from build123d import *

# Parameters (mm, degrees)
SKETCH_1_R           = 7.5
EXTRUDE_1_DEPTH      = 18
HOLE_WIZARD_M5_1_D   = 4.2
CUT_EXTRUDE_START    = -4
SKETCH_5_OUTSIDE_W   = 22.564
SKETCH_5_OUTSIDE_H   = 22.564
SKETCH_5_OUTSIDE_R   = 5
CUT_EXTRUDE_1_DEPTH  = 10.1
CHAMFER_1_SIZE       = 0.5
SKETCH_6_OUTSIDE_W   = 22.564
SKETCH_6_OUTSIDE_H   = 22.564
SKETCH_6_OUTSIDE_W_2 = 30.328855636
SKETCH_6_OUTSIDE_H_2 = 14
CUT_EXTRUDE_2_DEPTH  = 21.892582416


with BuildPart() as part:
    # 草图1 → 凸台-拉伸1 (new body)
    with BuildSketch(Plane(origin=(0, 0, 0), x_dir=(0, 0, -1), z_dir=(1, 0, 0))):
        Circle(SKETCH_1_R)
    extrude(amount=EXTRUDE_1_DEPTH)

    # M5 螺纹孔1 (through all)
    with Locations(Plane(origin=(18, 0, 0), x_dir=(0, 0, -1), z_dir=(1, 0, 0))):
        with Locations((0, 0)):
            Hole(HOLE_WIZARD_M5_1_D / 2)

    # 草图5 outside → 切除-拉伸1 (cut)
    with BuildSketch(Plane(origin=(18, 0, 0), x_dir=(0, 0, -1), z_dir=(1, 0, 0)).offset(CUT_EXTRUDE_START)):
        Rectangle(SKETCH_5_OUTSIDE_W, SKETCH_5_OUTSIDE_H)
        Circle(SKETCH_5_OUTSIDE_R, mode=Mode.SUBTRACT)
    extrude(amount=-CUT_EXTRUDE_1_DEPTH, mode=Mode.SUBTRACT)

    # 倒角1
    chamfer_1_edges = [part.edges().sort_by_distance(p)[0] for p in [
        (14, 0, 7.5),
        (3.9, 0, 7.5),
        (0, 0, 7.5),
        (18, 0, 7.5),
    ]]
    chamfer(chamfer_1_edges, length=CHAMFER_1_SIZE)

    # 草图6 outside → 切除-拉伸2 (cut, through all)
    with BuildSketch(Plane(origin=(18, 0, 0), x_dir=(0, 0, -1), z_dir=(1, 0, 0))):
        Rectangle(SKETCH_6_OUTSIDE_W, SKETCH_6_OUTSIDE_H)
        Rectangle(SKETCH_6_OUTSIDE_W_2, SKETCH_6_OUTSIDE_H_2, mode=Mode.SUBTRACT)
    extrude(amount=-CUT_EXTRUDE_2_DEPTH, mode=Mode.SUBTRACT)


solid = part.part
Read the model definition and answer for the solid it produces. Units are mm, in the model's axes. A direction names the side the tool comes from. Round coordinates to 2 decimals unless told otherwise and drop trailing zeros. Write each loop counter-clockwise with the first axis right and the second up, starting at its lowest first coordinate (ties: lowest second). Pieces come first, ordered by that corner, then holes.
1. The part is cut by section B-B, the plane x = 8. Determine the outline of the cut face in (y, z).
2. Given pin 1 Ø5 at (x, z) = (10, 2) entering from -Y; pin 2 Ø3 at (x, y) = (9, 2.5) entering from +Z; pin 3 Ø2 at (x, z) = (2, 5) entering from +Y, each flat-ended and moving along its own axis, determine where each tip first touches the part or whether it passes through.
3. Which of the six approach directions +Z, -Z, +X, -X, +Y, -Y give full straight-line access (tool end or side, diameter ignored) to faces 1 (the face through (14, 5, 2)), 2 (the face through (3.765, 0.157, -7.134)), 3 (the face through (14.14, -0.16, 7.14))?
4. Determine the mould class of faces 4 (the face through (0.135, 0.157, 7.134)), 5 (the face through (3.9, 5, 2)), 6 (the face through (2, -7, 0)) for opening direction X: pulls with the +X half, pulls with the -X half, needs draft (parallel to the pull), parting line crosses it, or undercut.
5. Straight lines are drawn through the part: L1, parallel to X at y = 4.25, z = -3.5; L2, parallel to Y at x = 10.25, z = 0; L3, parallel to Z at x = 17.25, y = 0.75. For each, find the intervals that lie inside material, in ascending order.
6. The part is cut by section A-A, the plane y = 0. Determine the outline of the cut face in (x, z), then the cut area to 3 significant figures.
Values:
1. outline: circle Ø10 at (0, 0); hole circle Ø4.2 at (0, 0)
2. pin 1: stops at y = -5
2. pin 2: stops at z = 4.9
2. pin 3: stops at y = 6.34
3. face 1: none
3. face 2: -Z
3. face 3: +Z
4. face 4: pulls with the -X half
4. face 5: undercut
4. face 6: needs draft
5. L1: x = 0 to 3.9, 14 to 18
5. L2: y = -5 to -2.1, 2.1 to 5
5. L3: z = -7.46 to -1.96, 1.96 to 7.46
6. outline: (0, -7) - (0.5, -7.5) - (3.4, -7.5) - (3.9, -7) - (3.9, -5) - (14, -5) - (14, -7) - (14.5, -7.5) - (17.5, -7.5) - (18, -7) - (18, -2.1) - (0, -2.1) - close; (0, 2.1) - (18, 2.1) - (18, 7) - (17.5, 7.5) - (14.5, 7.5) - (14, 7) - (14, 5) - (3.9, 5) - (3.9, 7) - (3.4, 7.5) - (0.5, 7.5) - (0, 7) - close
6. area: 143 mm2
